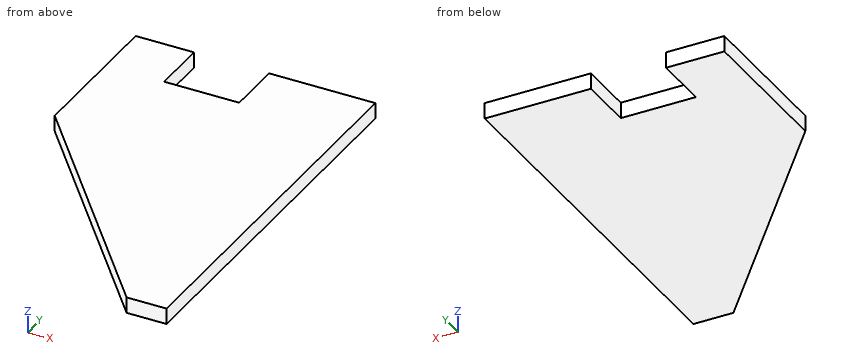
```python
from build123d import *

# Parameters (mm, degrees)
BOSS_EXTRUDE1_DEPTH = 20


with BuildPart() as part:
    # Sketch1 → Boss-Extrude1 (new body)
    with BuildSketch(Plane.XY):
        Polygon((0, 0), (0, -490), (-50, -490), (-300, -190), (-300, 0), (-227, 0), (-227, -70), (-133, -70), (-133, 0), align=None)
    extrude(amount=BOSS_EXTRUDE1_DEPTH)


solid = part.part
```
Can you work these out from the model? Positions are in its coordinate system, mm. Round coordinates to 2 decimals unless told otherwise and drop trailing zeros. Loops run counter-clockwise (first coordinate to the right, second up) from the corner with the lowest first, then second, coordinate; pieces in that order, holes last. Notation, with made-up numbers: M 73.5,51.25 L 80.5,51.25 A13 cw 80.5,58.25 Z; hole C 1.25,-8 d11. An arc over 180 degrees is marked long. Answer in a Markdown table with one row per item.
1. If we section it at A-A, the plane z = 16.75: Please give me the cut outline in (x, y).
Established:
| item | result |
|---|---|
| outline | M -300,-190 L -50,-490 L 0,-490 L 0,0 L -133,0 L -133,-70 L -227,-70 L -227,0 L -300,0 Z |
2. I'm going to push a flat-ended pin straight in: pin 1 Ø1 at (x, z) = (-213, 12) entering from -Y. Where does the tip first touch, or does it pass through?
Established:
| item | result |
|---|---|
| pin 1 | y = -295 |
3. Please list where these lines run through material, in increasing order: line 1 (X direction, y = -31, z = 11.5); line 2 (X direction, y = -206, z = 17); line 3 (Y direction, x = -50.5, z = 7.25). Write a range as from..to.
Established:
| item | result |
|---|---|
| line 1 | -300..-227, -133..0 |
| line 2 | -286.67..0 |
| line 3 | -489.4..0 |
4. If we section it at C-C, the plane y = -374.5: Please give me the cut outline in (x, z).
Established:
| item | result |
|---|---|
| outline | M -146.25,0 L 0,0 L 0,20 L -146.25,20 Z |
5. If we section it at B-B, the plane x = -198: Please give me the cut outline in (y, z), plus the area to 3 significant figures.
Established:
| item | result |
|---|---|
| outline | M -312.4,0 L -70,0 L -70,20 L -312.4,20 Z |
| area | 4,850 mm² |
